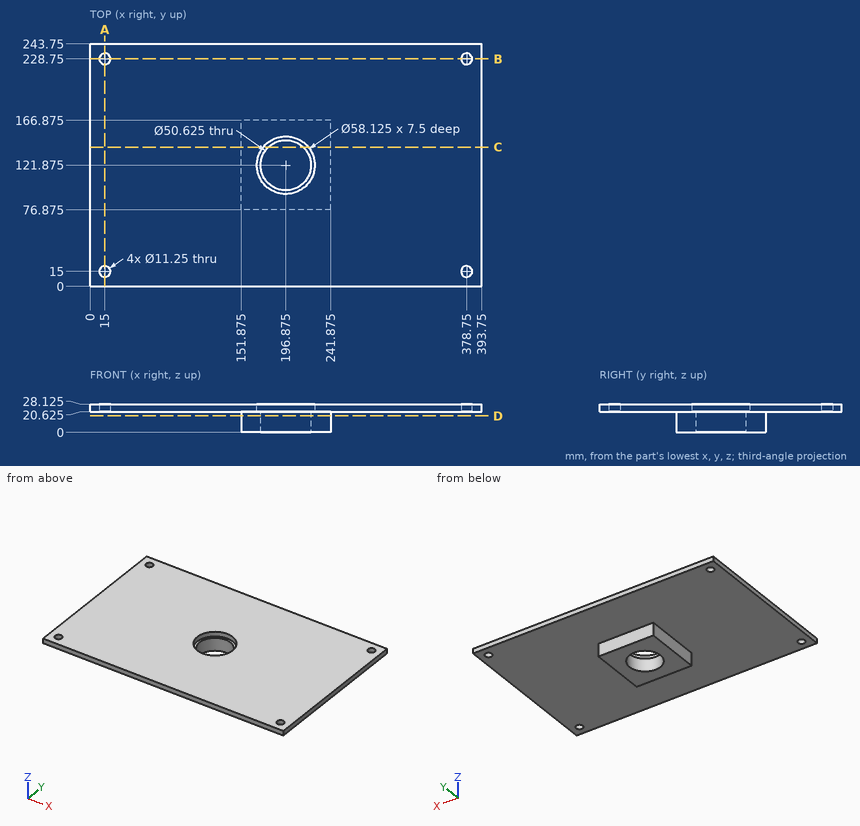
Job drawing, mm, ordinate dimensions from the low corner. One solid piece. Give positions to 0.01 mm unless a question says otherwise; leave off trailing zeros. Loops run counter-clockwise (first coordinate to the right, second up) from the corner with the lowest first, then second, coordinate; pieces in that order, holes last. Notation, with made-up numbers: M 25.5,60 L 49.5,60 A19 cw 49.5,77 Z; hole C 28,-29 d3. An arc over 180 degrees is marked long. Answer in a Markdown table with one row per item. Add a question column.
Item 1: Band-saw the part on B-B on y = 228.75. Give the cut face in (x, z) (3 decimals).
Item 2: Band-saw the part on C-C on y = 140. Give the cut face in (x, z) (3 decimals), then the cut area to 3 significant figures.
Item 3: Probe probe 1 along Y at (x, z) = (15, 25.75) (3 decimals); probe 2 along X at (y, z) = (166, 7.75) (3 decimals); probe 3 along Z at (x, y) = (112.5, 137.5) (3 decimals). List the from-to ranges inside material, lowest first.
Item 4: Band-saw the part on A-A on x = 15. Give the cut face in (y, z) (3 decimals), then the cut area to 3 significant figures.
Item 5: Band-saw the part on D-D on z = 16.5. Give the cut face in (x, y) (1 decimal).
Item 6: Drop flat-ended pins along their axis: P1, Ø10, axis at x = 378.75, y = 228.75, coming from the +Z side; P2, Ø10.5, axis at x = 211.5, z = 13, coming from the -Y side (3 decimals); P3, Ø10.5, axis at y = 141.5, z = 6, coming from the -X side (3 decimals); P4, Ø10, axis at x = 171.5, z = 4.5, coming from the +Y side (3 decimals). Give the stop position or say it passes through.
Reply:
| question | item | result |
|---|---|---|
| 1 | outline | M 0,20.625 L 9.375,20.625 L 9.375,28.125 L 0,28.125 Z; M 20.625,20.625 L 373.125,20.625 L 373.125,28.125 L 20.625,28.125 Z; M 384.375,20.625 L 393.75,20.625 L 393.75,28.125 L 384.375,28.125 Z |
| 2 | outline | M 0,20.625 L 151.875,20.625 L 151.875,0 L 179.206,0 L 179.206,20.625 L 174.157,20.625 L 174.157,28.125 L 0,28.125 Z; M 214.544,0 L 241.875,0 L 241.875,20.625 L 393.75,20.625 L 393.75,28.125 L 219.593,28.125 L 219.593,20.625 L 214.544,20.625 Z |
| 2 | area | 3,740 mm^2 |
| 3 | probe 1 | y = 0 to 9.375, 20.625 to 223.125, 234.375 to 243.75 |
| 3 | probe 2 | x = 151.875 to 241.875 |
| 3 | probe 3 | z = 20.625 to 28.125 |
| 4 | outline | M 0,20.625 L 9.375,20.625 L 9.375,28.125 L 0,28.125 Z; M 20.625,20.625 L 223.125,20.625 L 223.125,28.125 L 20.625,28.125 Z; M 234.375,20.625 L 243.75,20.625 L 243.75,28.125 L 234.375,28.125 Z |
| 4 | area | 1,660 mm^2 |
| 5 | outline | M 151.9,76.9 L 241.9,76.9 L 241.9,166.9 L 151.9,166.9 Z; hole C 196.9,121.9 d50.6 |
| 6 | P1 | passes through |
| 6 | P2 | stops at y = 76.875 |
| 6 | P3 | stops at x = 151.875 |
| 6 | P4 | stops at y = 166.875 |
